Here's how the part is built. I have some questions about the finished solid (model axes, mm). A direction names the side the tool comes from. Coordinates: 2 decimals unless noted, no trailing zeros. Write each loop counter-clockwise with the first axis right and the second up, starting at its lowest first coordinate (ties: lowest second). Pieces come first, ordered by that corner, then holes.
```python
from build123d import *

# Parameters (mm, degrees)
SKETCH_1_R          = 7.45
EXTRUDE_1_DEPTH     = 30
SKETCH_2_R          = 10
EXTRUDE_2_DEPTH     = 10
SKETCH_4_W          = 50
SKETCH_4_H          = 6
CUT_EXTRUDE_2_DEPTH = 5
CHAMFER_1_SIZE      = 1


with BuildPart() as part:
    # 草图1 → 凸台-拉伸1 (new body)
    with BuildSketch(Plane(origin=(0, 0, 0), x_dir=(1, 0, 0), z_dir=(0, 1, 0))):
        with Locations(Location((0, 0, 0), (0, 0, 270))):
            Circle(SKETCH_1_R)
    extrude(amount=-EXTRUDE_1_DEPTH)

    # 草图2 → 凸台-拉伸2 (add)
    with BuildSketch(Plane(origin=(0, 0, 0), x_dir=(1, 0, 0), z_dir=(0, 1, 0))):
        with Locations(Location((0, 0, 0), (0, 0, 270))):
            Circle(SKETCH_2_R)
    extrude(amount=EXTRUDE_2_DEPTH)

    # 草图4 → 切除-拉伸2 (cut)
    with BuildSketch(Plane(origin=(0, 10, 0), x_dir=(1, 0, 0), z_dir=(0, 1, 0))):
        Rectangle(SKETCH_4_W, SKETCH_4_H)
    extrude(amount=-CUT_EXTRUDE_2_DEPTH, mode=Mode.SUBTRACT)

    # 倒角1
    chamfer_1_edges = [part.edges().sort_by_distance(p)[0] for p in [
        (0, -30, -7.45),
    ]]
    chamfer(chamfer_1_edges, length=CHAMFER_1_SIZE)


solid = part.part
```
1) Imagine slicing it at D-D on y = -23. Please give me the cut outline in (x, z).
Values follow:
outline: circle Ø14.9 at (0, 0)
2) Imagine slicing it at B-B on x = 0. Please give me the cut outline in (y, z).
Values follow:
outline: (-30, -6.45) - (-29, -7.45) - (0, -7.45) - (0, -10) - (10, -10) - (10, -3) - (5, -3) - (5, 3) - (10, 3) - (10, 10) - (0, 10) - (0, 7.45) - (-29, 7.45) - (-30, 6.45) - close
3) On a 3-axis mill with a long thin cutter (end or side, diameter ignored), from which of +Z, -Z, +X, -X, +Y, -Y can I reach the whole of each face in a straight line? I mean faces 1 (the face through (0, 10, -6)), 2 (the face through (0, 8, -3)). Say none if no direction works.
Values follow:
face 1: +Z, -Z, +X, -X, +Y
face 2: +X, -X, +Y
4) Imagine slicing it at C-C on x = -8. Please give me the cut outline in (y, z), then the cut area to 3 significant figures.
Values follow:
outline: (0, -6) - (10, -6) - (10, -3) - (5, -3) - (5, 3) - (10, 3) - (10, 6) - (0, 6) - close
area: 90.0 mm2
5) Will these pins go through, and if not, where does the flat tip stop? pin 1 (5 mm diameter, centred on x = -5, z = 1.5, fed in from +Y); pin 2 (1 mm diameter, centred on y = -8, z = 6, fed in from -X); pin 3 (1.5 mm diameter, centred on y = -8.5, z = -7, fed in from +X); pin 4 (1.5 mm diameter, centred on x = -2, y = 7.5, fed in from -Z).
Values follow:
pin 1: stops at y = 10
pin 2: stops at x = -5.03
pin 3: stops at x = 4.05
pin 4: stops at z = -9.92
6) Imagine slicing it at A-A on z = 0. Please give me the cut outline in (x, y).
Values follow:
outline: (-10, 0) - (-7.45, 0) - (-7.45, -29) - (-6.45, -30) - (6.45, -30) - (7.45, -29) - (7.45, 0) - (10, 0) - (10, 5) - (-10, 5) - close
7) I need wall thicknesses on probe 1 along Y at (x, z) = (7.5, -5.75); probe 2 along Z at (x, y) = (-8.25, 7); probe 3 along Y at (x, z) = (9, 1.75). Which ranges of each line are inside material? Lowest first, please.
Values follow:
probe 1: y = 0 to 10
probe 2: z = -5.65 to -3, 3 to 5.65
probe 3: y = 0 to 5
8) We'd pull the mould along Z, two halves only. Please class faces 3 (the face through (0, 8, 3)), 4 (the face through (7.5, 0, -1.5)), 5 (the face through (-6.61, -14.3, 3.44)): pulls with the +Z half, pulls with the -Z half, needs draft (parallel to the pull), parting line crosses it, or undercut.
Values follow:
face 3: undercut
face 4: needs draft
face 5: parting line crosses it
